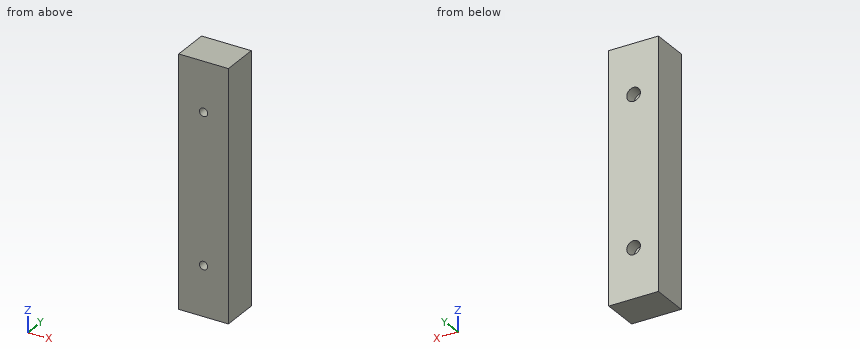
```python
from build123d import *

# Parameters (mm, degrees)
SKETCH_1_W                = 40
SKETCH_1_H                = 200
EXTRUDE_1_DEPTH           = 15
HOLE_WIZARD_1_D           = 6.6
HOLE_WIZARD_1_CBORE_D     = 11
HOLE_WIZARD_1_CBORE_DEPTH = 10


with BuildPart() as part:
    # 草图1 → 凸台-拉伸1 (new, symmetric)
    with BuildSketch(Plane(origin=(0, 0, 0), x_dir=(1, 0, 0), z_dir=(0, 1, 0))):
        Rectangle(SKETCH_1_W, SKETCH_1_H)
    extrude(amount=EXTRUDE_1_DEPTH, both=True)

    # 打孔尺寸(%根据)内六角圆柱头螺钉的类型1 (through all)
    with Locations(Plane(origin=(0, 15, 0), x_dir=(1, 0, 0), z_dir=(0, 1, 0))):
        with Locations((0, 60), (0, -60)):
            CounterBoreHole(HOLE_WIZARD_1_D / 2, HOLE_WIZARD_1_CBORE_D / 2, HOLE_WIZARD_1_CBORE_DEPTH)


solid = part.part
```
For this review, take the finished solid that the model builds, in its own axes (mm). Round coordinates to 2 decimals unless told otherwise and drop trailing zeros. Loops run counter-clockwise (first coordinate to the right, second up) from the corner with the lowest first, then second, coordinate; pieces in that order, holes last.
Q1. To check wall thickness, follow line 1 along Z through (x, y) = (0, 10.5); line 2 along Z through (x, y) = (4, 5.25); line 3 along X through (y, z) = (10.75, 60). State the ranges of each line that lie inside material, in increasing order.
Result sheet:
line 1: z = -100 to -65.5, -54.5 to 54.5, 65.5 to 100
line 2: z = -100 to -63.77, -56.23 to 56.23, 63.77 to 100
line 3: x = -20 to -5.5, 5.5 to 20
Q2. Insertion check: pin 1 Ø8.5 at (x, z) = (0, -60) entering from -Y; pin 2 Ø3.5 at (x, z) = (2.5, 61.5) entering from +Y. Each pin has a flat end and moves straight along its axis. Give the tip position at first contact, or say it passes through.
Result sheet:
pin 1: stops at y = -15
pin 2: stops at y = 5
Q3. Add section B-B on z = 60. Write out the cut boundary in (x, y).
Result sheet:
outline: (-20, -15) - (-3.3, -15) - (-3.3, 5) - (-5.5, 5) - (-5.5, 15) - (-20, 15) - close; (3.3, -15) - (20, -15) - (20, 15) - (5.5, 15) - (5.5, 5) - (3.3, 5) - close
Q4. Add section A-A on x = 0. Write out the cut boundary in (y, z), plus the area to 3 significant figures.
Result sheet:
outline: (-15, -100) - (15, -100) - (15, -65.5) - (5, -65.5) - (5, -63.3) - (-15, -63.3) - close; (-15, -56.7) - (5, -56.7) - (5, -54.5) - (15, -54.5) - (15, 54.5) - (5, 54.5) - (5, 56.7) - (-15, 56.7) - close; (-15, 63.3) - (5, 63.3) - (5, 65.5) - (15, 65.5) - (15, 100) - (-15, 100) - close
area: 5,520 mm2
